Check sheet for the drawn part. Datum: minimum x, y, z corner. Units: mm. A direction names the side the tool comes from. Coordinates: 2 decimals unless noted, no trailing zeros. Write each loop counter-clockwise with the first axis right and the second up, starting at its lowest first coordinate (ties: lowest second). Pieces come first, ordered by that corner, then holes. Notation, with made-up numbers: M 69,44.5 L 101,44.5 A22 ccw 101,71.5 Z; hole C -14,52 d6. An arc over 180 degrees is marked long. Answer as CSV lines item,"result".
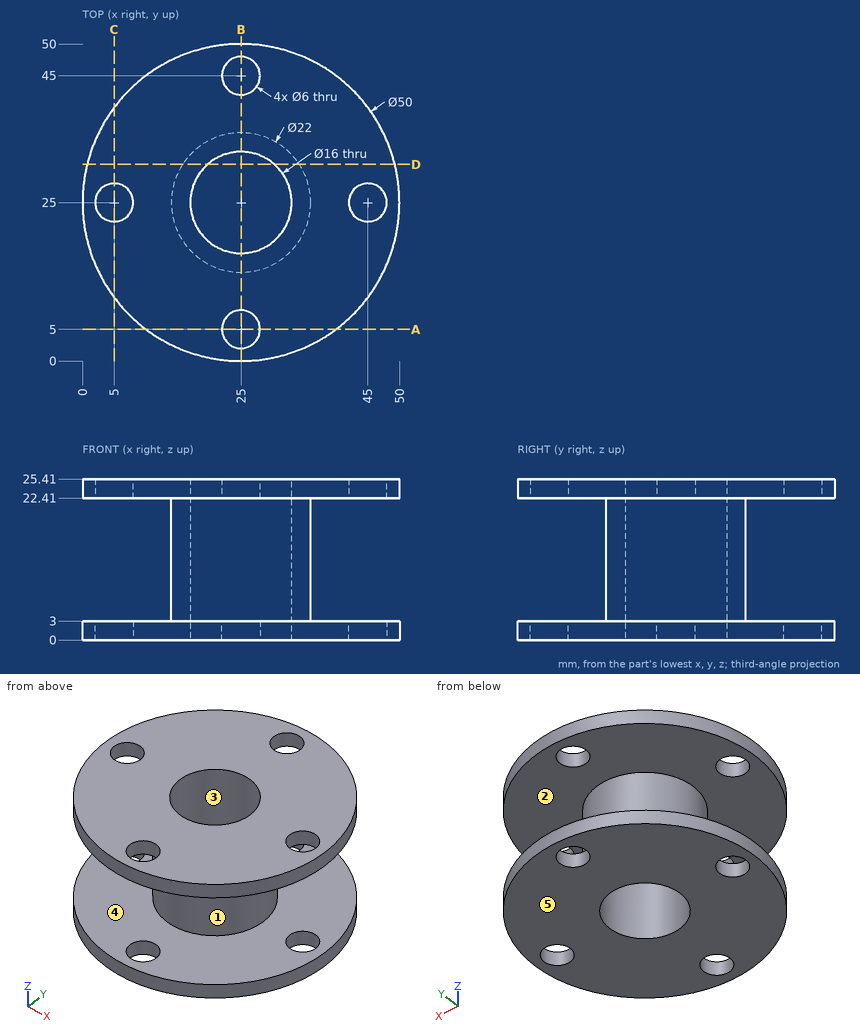
1) Section check D-D, the plane y = 31. Record the boundary of the cut face in (x, z).
Answer key:
outline,"M 0.73,0 L 19.71,0 L 19.71,25.41 L 0.73,25.41 L 0.73,22.41 L 15.78,22.41 L 15.78,3 L 0.73,3 Z; M 30.29,0 L 49.27,0 L 49.27,3 L 34.22,3 L 34.22,22.41 L 49.27,22.41 L 49.27,25.41 L 30.29,25.41 Z"
2) Section check B-B, the plane x = 25. Give the number of separate pieces and of enclosed holes in the cut face, plus the area to 3 significant figures.
Answer key:
separate pieces,"6"
enclosed holes,"0"
area,"248 mm2"
3) Mould release check, pull along Y, two halves, no side actions. Record for the marked faces 1, 2 and 3: pulls with the +Y half, pulls with the -Y half, needs draft (parallel to the pull), parting line crosses it, or undercut.
Answer key:
face 1,"parting line crosses it"
face 2,"needs draft"
face 3,"undercut"
4) Section check A-A, the plane y = 5. Record the boundary of the cut face in (x, z), plus the area to 3 significant figures.
Answer key:
outline,"M 10,0 L 22,0 L 22,3 L 10,3 Z; M 10,22.41 L 22,22.41 L 22,25.41 L 10,25.41 Z; M 28,0 L 40,0 L 40,3 L 28,3 Z; M 28,22.41 L 40,22.41 L 40,25.41 L 28,25.41 Z"
area,"144 mm2"
5) Depth check by flat-ended pin: P1, Ø1, axis at x = 17, z = 10, coming from the +Y side; P2, Ø5, axis at x = 25, y = 45, coming from the +Z side; P3, Ø6, axis at x = 34.5, z = 10.5, coming from the -Y side; P4, Ø8, axis at y = 32.5, z = 13.5, coming from the +X side. Enter the tip coordinate at first touch or a pass-through.
Answer key:
P1,"stops at y = 33.05"
P2,"passes through"
P3,"stops at y = 16.13"
P4,"stops at x = 35.43"
6) Thickness scan on line 1 along Y through (x, z) = (25, 1.6); line 2 along Z through (x, y) = (5, 29.5); line 3 along Y through (x, z) = (25, 18.5). Record the ranges inside material, lowest first.
Answer key:
line 1,"y = 0 to 2, 8 to 17, 33 to 42, 48 to 50"
line 2,"z = 0 to 3, 22.41 to 25.41"
line 3,"y = 14 to 17, 33 to 36"
7) Tool access check on the marked faces 4 and 5. Record the directions out of +Z, -Z, +X, -X, +Y, -Y that give a thin tool (end or side, any length) a straight path to the whole face; none if there is none.
Answer key:
face 4,"none"
face 5,"-Z, +X, -X, +Y, -Y"
